Can you work these out from the model? Positions are in its coordinate system, mm. A direction names the side the tool comes from. Give positions to 0.01 mm unless a question says otherwise; leave off trailing zeros. Loops run counter-clockwise (first coordinate to the right, second up) from the corner with the lowest first, then second, coordinate; pieces in that order, holes last. Notation, with made-up numbers: M 88,-33.75 L 123,-33.75 A20 cw 123,-26.75 Z; hole C 11,-18 d10. An arc over 180 degrees is marked long. Use CSV: the item, a comma, the result in double quotes.
from build123d import *

# Parameters (mm, degrees)
SKETCH1_W           = 227
SKETCH1_H           = 200
BOSS_EXTRUDE1_DEPTH = 14
SKETCH2_R           = 65
BOSS_EXTRUDE2_DEPTH = 6
SKETCH3_R           = 70
BOSS_EXTRUDE3_DEPTH = 8


with BuildPart() as part:
    # Sketch1 → Boss-Extrude1 (new body)
    with BuildSketch(Plane.XY):
        with Locations((113.5, 100)):
            Rectangle(SKETCH1_W, SKETCH1_H)
    extrude(amount=BOSS_EXTRUDE1_DEPTH)

    # Sketch2 → Boss-Extrude2 (add)
    with BuildSketch(Plane.XY.offset(14)):
        with Locations(Location((113.5, 100, 0), (0, 0, 180))):
            Circle(SKETCH2_R)
    extrude(amount=BOSS_EXTRUDE2_DEPTH)

    # Sketch3 → Boss-Extrude3 (add)
    with BuildSketch(Plane(origin=(0, 0, 0), x_dir=(-1, 0, 0), z_dir=(0, 0, -1))):
        with Locations((-113.5, 100)):
            Circle(SKETCH3_R)
    extrude(amount=BOSS_EXTRUDE3_DEPTH)


solid = part.part
Q1. I want a section at C-C, the plane z = -4.5. Please give me the cut outline in (x, y), then the cut area to 3 significant figures.
Model answer:
outline,"C 113.5,100 d140"
area,"15,400 mm2"
Q2. I want a section at D-D, the plane y = 22. Please give me the cut outline in (x, z), then the cut area to 3 significant figures.
Model answer:
outline,"M 0,0 L 227,0 L 227,14 L 0,14 Z"
area,"3,180 mm2"
Q3. For faces 1 (the flat face through (111.9, 34.7, 14)), 2 (the flat face through (227, 99, 7)), 3 (the cylindrical face through (122.613, 169.404, -3.944)), which set-ups out of +Z, -Z, +X, -X, +Y, -Y let a thin tool reach every point of the face, with its end or its side?
Model answer:
face 1,"+Z"
face 2,"+Z, -Z, +X, +Y, -Y"
face 3,"-Z"
Q4. I want a section at A-A, the plane x = 113.5. Please give me the cut outline in (y, z), then the cut area to 3 significant figures.
Model answer:
outline,"M 0,0 L 30,0 L 30,-8 L 170,-8 L 170,0 L 200,0 L 200,14 L 165,14 L 165,20 L 35,20 L 35,14 L 0,14 Z"
area,"4,700 mm2"
Q5. Please list where these lines run through material, in increasing order: L1, parallel to Z at x = 181.5, y = 171; L2, parallel to Z at x = 99.5, y = 32.5; L3, parallel to X at y = 135, z = -6.5. Write a range as from..to.
Model answer:
L1,"0..14"
L2,"-8..14"
L3,"52.88..174.12"
Q6. I want a section at B-B, the plane y = 100. Please give me the cut outline in (x, z), then the cut area to 3 significant figures.
Model answer:
outline,"M 0,0 L 43.5,0 L 43.5,-8 L 183.5,-8 L 183.5,0 L 227,0 L 227,14 L 178.5,14 L 178.5,20 L 48.5,20 L 48.5,14 L 0,14 Z"
area,"5,080 mm2"
Q7. I'm going to push flat-ended pins straight in: P1, Ø5, axis at x = 129.5, z = -3, coming from the +Y side; P2, Ø2, axis at x = 32.5, y = 90.5, coming from the +Z side; P3, Ø5, axis at x = 60, z = -3, coming from the -Y side; P4, Ø3, axis at y = 151.5, z = 0.5, coming from the -X side. Where does each tip first touch, or does it pass through?
Model answer:
P1,"y = 168.69"
P2,"z = 14"
P3,"y = 52.05"
P4,"x = 0"
